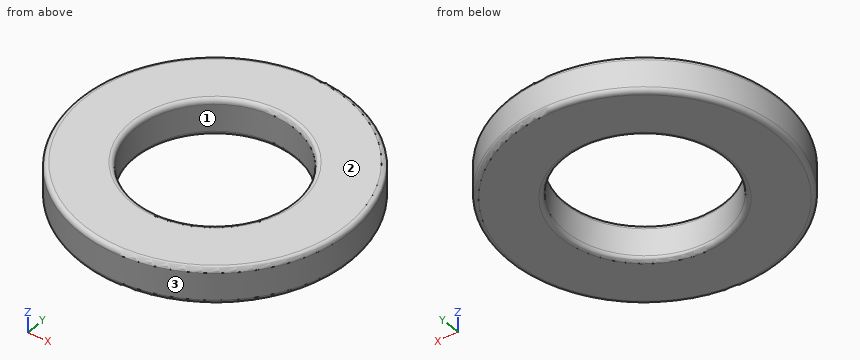
from build123d import *

# Parameters (mm, degrees)
SKETCH_1_R      = 30
SKETCH_1_R_2    = 17.5
EXTRUDE_1_DEPTH = 8
FILLET_1_R      = 1


with BuildPart() as part:
    # 草图1 → 凸台-拉伸1 (new body)
    with BuildSketch(Plane.XY):
        Circle(SKETCH_1_R)
        Circle(SKETCH_1_R_2, mode=Mode.SUBTRACT)
    extrude(amount=EXTRUDE_1_DEPTH)

    # 圆角1
    fillet_1_edges = [part.edges().sort_by_distance(p)[0] for p in [
        (-30, 0, 0),
        (-30, 0, 8),
        (-17.5, 0, 0),
        (-17.5, 0, 8),
    ]]
    fillet(fillet_1_edges, radius=FILLET_1_R)


solid = part.part
Work out the finished part from the listing and answer in its coordinate system (mm). Face numbers are marked on the shaded views. Give positions to 0.01 mm unless a question says otherwise; leave off trailing zeros. Order: outer loops, then holes, each group sorted by start corner. A loop starts at its lowest first (then second) coordinate and runs counter-clockwise, first axis right, second up. Notation, with made-up numbers: (72.25, -7.75) -> (76.25, -7.75) arc R13 cw to (76.25, 16.25) -> close; hole circle Ø5 at (41, 31). An arc over 180 degrees is marked (long way). One line per item, written item: value.
Item 1: Flat-ended cylindrical pins translate along their axes: P1, Ø5, axis at x = -5, y = 14.5, coming from the -Z side; P2, Ø1, axis at x = 9.5, z = 5.5, coming from the +Y side. Find the tip coordinate at first contact, or state that the pin passes through.
Answer sheet:
P1: z = 0.25
P2: y = 28.62
Item 2: Find section C-C, the plane z = 4.5. Give the vertices of the cut face in (x, y).
Answer sheet:
outline: circle Ø60 at (0, 0); hole circle Ø35 at (0, 0)
Item 3: Determine the mould class of the marked faces 1, 2 and 3 for opening direction Y: released by +Y, released by -Y, zero draft, split by the parting line, or undercut.
Answer sheet:
face 1: undercut
face 2: zero draft
face 3: split by the parting line
Item 4: Find section A-A, the plane x = 0. Give the vertices of the cut face in (y, z), plus the area to 3 significant figures.
Answer sheet:
outline: (-30, 1) arc R1 ccw to (-29, 0) -> (-18.5, 0) arc R1 ccw to (-17.5, 1) -> (-17.5, 7) arc R1 ccw to (-18.5, 8) -> (-29, 8) arc R1 ccw to (-30, 7) -> close; (17.5, 1) arc R1 ccw to (18.5, 0) -> (29, 0) arc R1 ccw to (30, 1) -> (30, 7) arc R1 ccw to (29, 8) -> (18.5, 8) arc R1 ccw to (17.5, 7) -> close
area: 198 mm²
Item 5: Straight lines are drawn through the part: probe 1 along Y at (x, z) = (0, 4.1); probe 2 along X at (y, z) = (-5, 7.25); probe 3 along Y at (x, z) = (6, 6.75). For each, find the intervals that lie inside material, in ascending order.
Answer sheet:
probe 1: -30 to -17.5, 17.5 to 30
probe 2: -29.55 to -16.8, 16.8 to 29.55
probe 3: -29.39 to -16.44, 16.44 to 29.39
